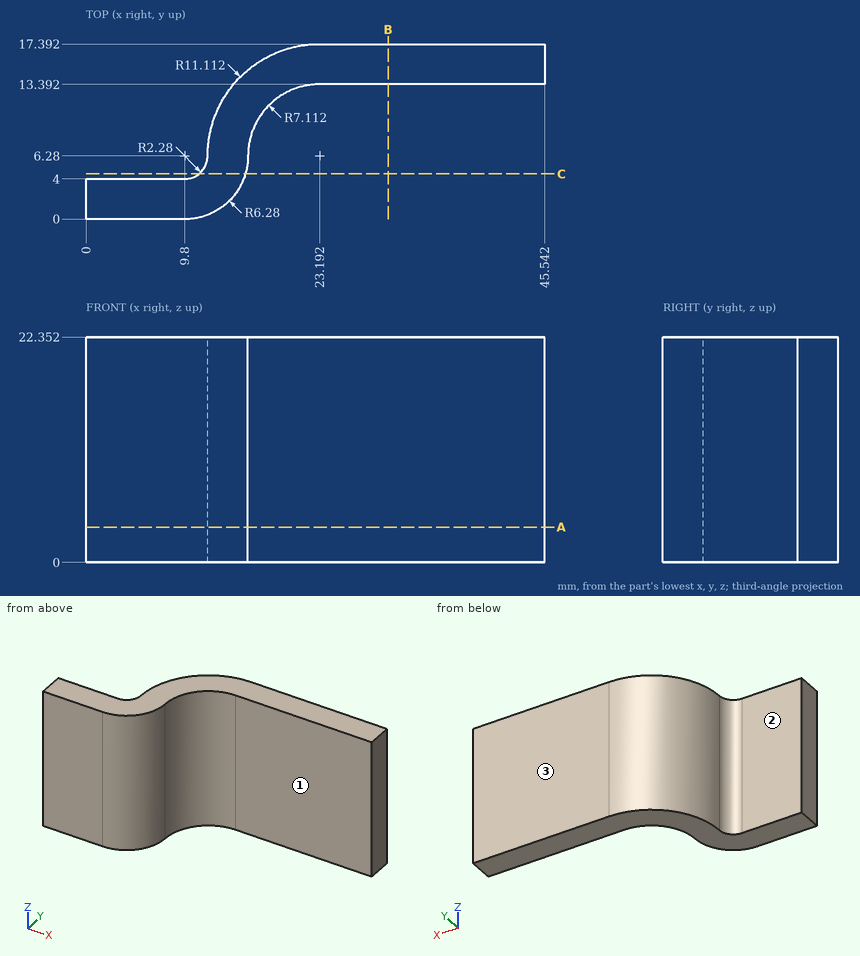
Geometry: see drawing. Coordinates: mm, zero at the bounding-box minimum. A direction names the side the tool comes from. Give positions to 0.01 mm unless a question says otherwise; leave off trailing zeros. Order: outer loops, then holes, each group sorted by start corner. A loop starts at its lowest first (then second) coordinate and runs counter-clockwise, first axis right, second up. Notation, with made-up numbers: (-16.5, 74) - (18.5, 74) arc R27 cw to (18.5, 101) - close; hole circle Ø11 at (72.25, 16.5). An arc over 180 degrees is marked (long way). Use CSV: the item, a comma, the result in double quotes.
1. Access query for the marked faces 1, 2 and 3. Directions: +Z, -Z, +X, -X, +Y, -Y. A direction counts if a zero-diameter tool reaches every point of the face in a straight line with its end or side. Return the directions, or none.
Answers below:
face 1,"+Z, -Z, +X, -Y"
face 2,"+Z, -Z, -X, +Y"
face 3,"+Z, -Z, +X, -X, +Y"
2. Section query A-A (z = 3.5). Output: boundary loops of the cut face in (x, y).
Answers below:
outline,"(0, 0) - (9.8, 0) arc R6.28 ccw to (16.08, 6.28) arc R7.11 cw to (23.19, 13.39) - (45.54, 13.39) - (45.54, 17.39) - (23.19, 17.39) arc R11.11 ccw to (12.08, 6.28) arc R2.28 cw to (9.8, 4) - (0, 4) - close"
3. Contact query for flat-ended pins moving along their axis: pin 1 (6.5 mm diameter, centred on x = 40, z = 9.5, fed in from -Y); pin 2 (3 mm diameter, centred on x = 3.5, z = 9, fed in from +Y); pin 3 (1.5 mm diameter, centred on y = 8.5, z = 8, fed in from +X). Output: stop coordinate, or through.
Answers below:
pin 1,"y = 13.39"
pin 2,"y = 4"
pin 3,"x = 16.73"
4. Material intervals for line 1 along Y through (x, z) = (40, 21); line 2 along Y through (x, z) = (5, 11.5); line 3 along X through (y, z) = (7, 19.5), sorted ascending. Write a range as from..to.
Answers below:
line 1,"13.39..17.39"
line 2,"0..4"
line 3,"12.1..16.12"
5. Section query B-B (x = 30). Output: boundary loops of the cut face in (y, z).
Answers below:
outline,"(13.39, 0) - (17.39, 0) - (17.39, 22.35) - (13.39, 22.35) - close"
6. Section query C-C (y = 4.5). Output: boundary loops of the cut face in (x, z), plus the area to 3 significant figures.
Answers below:
outline,"(11.22, 0) - (15.82, 0) - (15.82, 22.35) - (11.22, 22.35) - close"
area,"103 mm2"
